Geometry: final body of the model. Coordinates: model frame, mm. Round coordinates to 2 decimals unless told otherwise and drop trailing zeros. Loops run counter-clockwise (first coordinate to the right, second up) from the corner with the lowest first, then second, coordinate; pieces in that order, holes last. Notation, with made-up numbers: (35.25, -33.75) - (68.25, -33.75) arc R7 cw to (68.25, -23.75) - close; hole circle Ø3 at (-14.75, 41). An arc over 180 degrees is marked (long way). Answer as CSV lines item,"result".
from build123d import *

# Parameters (mm, degrees)
SKETCH_1_R      = 9
EXTRUDE_1_DEPTH = 14


with BuildPart() as part:
    # 草图1 → 凸台-拉伸1 (new body)
    with BuildSketch(Plane.XY):
        Polygon((0, 0), (0, 100), (115, 100), (115, 125), (485, 125), (485, 100), (600, 100), (600, 0), align=None)
        with Locations((240, 65)):
            Circle(SKETCH_1_R, mode=Mode.SUBTRACT)
        with Locations((440, 65)):
            Circle(SKETCH_1_R, mode=Mode.SUBTRACT)
    extrude(amount=EXTRUDE_1_DEPTH)


solid = part.part
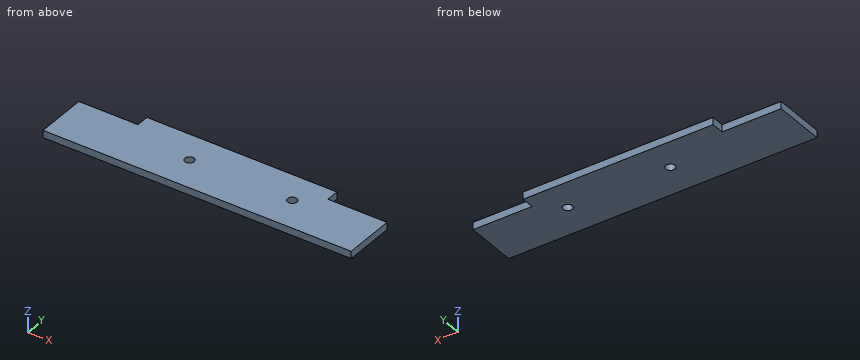
(1) Section D-D (x = 438.5). Output: boundary loops of the cut face in (y, z).
Findings below:
outline,"(0, 0) - (56.13, 0) - (56.13, 14) - (0, 14) - close; (73.87, 0) - (125, 0) - (125, 14) - (73.87, 14) - close"
(2) Section A-A (x = 240). Output: boundary loops of the cut face in (y, z), and give its area (3 significant figures).
Findings below:
outline,"(0, 0) - (56, 0) - (56, 14) - (0, 14) - close; (74, 0) - (125, 0) - (125, 14) - (74, 14) - close"
area,"1,500 mm2"
(3) Section B-B (y = 65). Output: boundary loops of the cut face in (x, z), and give its area (3 significant figures).
Findings below:
outline,"(0, 0) - (231, 0) - (231, 14) - (0, 14) - close; (249, 0) - (431, 0) - (431, 14) - (249, 14) - close; (449, 0) - (600, 0) - (600, 14) - (449, 14) - close"
area,"7,900 mm2"
(4) Material intervals for line 1 along Y through (x, z) = (240, 11); line 2 along Y through (x, z) = (36, 11.5); line 3 along Y through (x, z) = (242.5, 8.75), sorted ascending.
Findings below:
line 1,"0 to 56, 74 to 125"
line 2,"0 to 100"
line 3,"0 to 56.35, 73.65 to 125"
(5) Section C-C (z = 7). Output: boundary loops of the cut face in (x, y).
Findings below:
outline,"(0, 0) - (600, 0) - (600, 100) - (485, 100) - (485, 125) - (115, 125) - (115, 100) - (0, 100) - close; hole circle Ø18 at (240, 65); hole circle Ø18 at (440, 65)"
(6) Pin query (flat end, axial travel): P1, Ø1.5, axis at x = 127, y = 33, coming from the -Z side; P2, Ø4, axis at y = 106.5, z = 9, coming from the +X side; P3, Ø4, axis at x = 83.5, z = 4, coming from the +Y side. Return the tip coordinate at first contact, or that it passes through.
Findings below:
P1,"z = 0"
P2,"x = 485"
P3,"y = 100"
